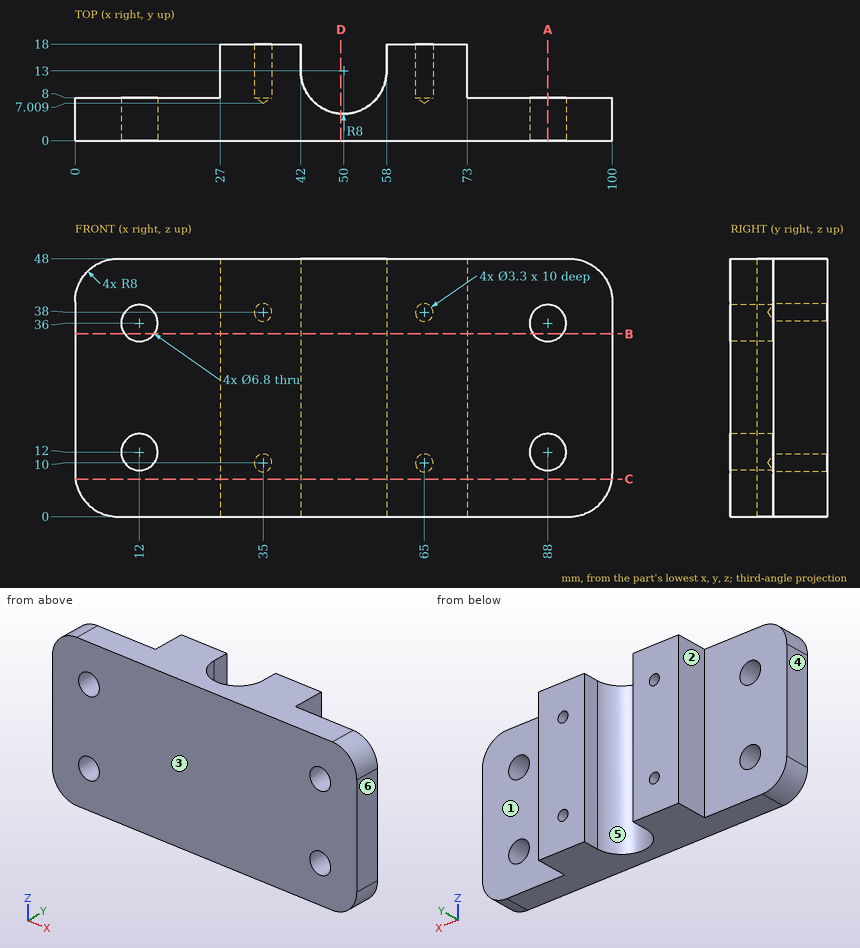
Here's the drawing with two shaded views (mm, measured from the low corner). I have some questions. A direction names the side the tool comes from. Give positions to 0.01 mm unless a question says otherwise; leave off trailing zeros. Loops run counter-clockwise (first coordinate to the right, second up) from the corner with the lowest first, then second, coordinate; pieces in that order, holes last. Notation, with made-up numbers: M 7.25,-6 L 20.25,-6 A28 cw 20.25,15 Z; hole C -15.5,85.25 d8. An arc over 180 degrees is marked long. One line per item, written item: value. Start each with the question number.
1) I'm going to push flat-ended pins straight in: pin 1 (5.5 mm diameter, centred on x = 12, z = 36, fed in from -Y); pin 2 (5.5 mm diameter, centred on y = 14.5, z = 13, fed in from -X); pin 3 (3 mm diameter, centred on y = 11.5, z = 17.5, fed in from +X); pin 4 (8 mm diameter, centred on x = 82.5, z = 34, fed in from +Y). Where does each tip first touch, or does it pass through?
2) If I drill on line 1 (Z direction, x = 35, y = 13.25); line 2 (Z direction, x = 88, y = 6.25); line 3 (X direction, y = 15, z = 38), over which ranges is the centre line in solid material (lowest first)? Write a range as [from, to].
3) If we section it at C-C, the plane z = 7: Write out the boundary of the cut face in (x, y).
4) If we section it at A-A, the plane x = 88: Write out the boundary of the cut face in (y, z).
5) Thinking about a two-plate mould opening in X: for the marked faces 4, 5 and 6, which applies, +X half, -X half, draft (parallel to the pull), parting line (faces both ways), or undercut?
6) If we section it at B-B, the plane z = 34: Write out the boundary of the cut face in (x, y).
7) If we section it at D-D, the plane x = 49.5: Write out the boundary of the cut face in (y, z) (1 decimal), and give its area (3 significant figures).
8) On a 3-axis mill with a long thin cutter (end or side, diameter ignored), from which of +Z, -Z, +X, -X, +Y, -Y can I reach the whole of each face in a straight line? I mean the marked faces 1, 2 and 3. Say none if no direction works.
Completed:
1. pin 1: passes through
1. pin 2: stops at x = 27
1. pin 3: stops at x = 73
1. pin 4: stops at y = 8
2. line 1: z = [0, 8.35], [11.65, 36.35], [39.65, 48]
2. line 2: z = [0, 8.6], [15.4, 32.6], [39.4, 48]
2. line 3: x = [27, 33.35], [36.65, 42], [58, 63.35], [66.65, 73]
3. outline: M 0.06,0 L 99.94,0 L 99.94,8 L 73,8 L 73,18 L 58,18 L 58,13 A8 cw 42,13 L 42,18 L 27,18 L 27,8 L 0.06,8 Z
4. outline: M 0,0 L 8,0 L 8,8.6 L 0,8.6 Z; M 0,15.4 L 8,15.4 L 8,32.6 L 0,32.6 Z; M 0,39.4 L 8,39.4 L 8,48 L 0,48 Z
5. face 4: -X half
5. face 5: undercut
5. face 6: +X half
6. outline: M 0,0 L 9.25,0 L 9.25,8 L 0,8 Z; M 14.75,0 L 85.25,0 L 85.25,8 L 73,8 L 73,18 L 58,18 L 58,13 A8 cw 42,13 L 42,18 L 27,18 L 27,8 L 14.75,8 Z; M 90.75,0 L 100,0 L 100,8 L 90.75,8 Z
7. outline: M 0,0 L 5,0 L 5,48 L 0,48 Z
7. area: 241 mm^2
8. face 1: +Z, -Z, +X, +Y
8. face 2: +Z, -Z, -X, +Y
8. face 3: +Z, -Z, +X, -X, -Y
